```python
from build123d import *

# Parameters (mm, degrees)
BOSS_EXTRUDE1_DEPTH                                 = 8
CBORE_FOR_M3_HEX_SOCKET_HEAD_CAP_SCREW1_D           = 3.4
CBORE_FOR_M3_HEX_SOCKET_HEAD_CAP_SCREW1_CBORE_D     = 6.5
CBORE_FOR_M3_HEX_SOCKET_HEAD_CAP_SCREW1_CBORE_DEPTH = 3.4


with BuildPart() as part:
    # Sketch1 → Boss-Extrude1 (new body)
    with BuildSketch(Plane.XY):
        with BuildLine():
            Line((-27.5, 4), (27.5, 4))
            ThreePointArc((27.5, 4), (31.5, 0), (27.5, -4))
            Line((27.5, -4), (-27.5, -4))
            ThreePointArc((-27.5, -4), (-31.5, 0), (-27.5, 4))
        make_face()
    extrude(amount=BOSS_EXTRUDE1_DEPTH)

    # CBORE for M3 Hex Socket Head Cap Screw1 (through all)
    with Locations(Plane.XY.offset(8)):
        with Locations((-20, 0), (20, 0)):
            CounterBoreHole(CBORE_FOR_M3_HEX_SOCKET_HEAD_CAP_SCREW1_D / 2, CBORE_FOR_M3_HEX_SOCKET_HEAD_CAP_SCREW1_CBORE_D / 2, CBORE_FOR_M3_HEX_SOCKET_HEAD_CAP_SCREW1_CBORE_DEPTH)


solid = part.part
```
Design review of the part built by this model. Coordinates are the model's own, in mm. A direction names the side the tool comes from. Coordinates: 2 decimals unless noted, no trailing zeros. Order: outer loops, then holes, each group sorted by start corner. A loop starts at its lowest first (then second) coordinate and runs counter-clockwise, first axis right, second up. Notation, with made-up numbers: M 31.25,54 L 87.25,54 A19 cw 87.25,59 Z; hole C 33.5,70.5 d5. An arc over 180 degrees is marked long. Answer as a JSON object with one key per item and string values. Group by question number.
1) Add section B-B, the plane y = 0. Write out the cut boundary in (x, z).
2) Wall thickness on L1, parallel to Y at x = -20, z = 6.1; L2, parallel to X at y = 2.5, z = 6.25; L3, parallel to Y at x = 20, z = 2.05: over which ranges is each line inside the solid? List them lowest first.
3) Tool access review of faces 4 (the cylindrical face through (16.753, 0.143, 6.324)), 5 (the cylindrical face through (18.43, -0.65, 2.27)): name each direction out of +Z, -Z, +X, -X, +Y, -Y from which nothing blocks a thin tool from reaching the whole face with its end or side.
4) Add section A-A, the plane x = 20. Write out the cut boundary in (y, z).
5) For pin 1 (4 mm diameter, centred on x = -20, y = 0, fed in from +Z), flat-tipped, find the tip position at first contact; note if it passes through.
6) Add section C-C, the plane z = 3.5. Write out the cut boundary in (x, y), then the cut area to 3 significant figures.
7) Mouldability with a two-part tool opening along X and no side actions: class faces 1 (the cylindrical face through (31.5, 0.1, 3.9)), 2 (the flat face through (21.4, -1.4, 4.6)), 3 (the flat face through (0, 0, 8)) as pulls with the +X half, pulls with the -X half, needs draft (parallel to the pull), parting line crosses it, or undercut.
Computed values:
{
 "1": {"outline": "M -31.5,0 L -21.7,0 L -21.7,4.6 L -23.25,4.6 L -23.25,8 L -31.5,8 Z; M -18.3,0 L 18.3,0 L 18.3,4.6 L 16.75,4.6 L 16.75,8 L -16.75,8 L -16.75,4.6 L -18.3,4.6 Z; M 21.7,0 L 31.5,0 L 31.5,8 L 23.25,8 L 23.25,4.6 L 21.7,4.6 Z"},
 "2": {"L1": "y = -4 to -3.25, 3.25 to 4", "L2": "x = -30.62 to -22.08, -17.92 to 17.92, 22.08 to 30.62", "L3": "y = -4 to -1.7, 1.7 to 4"},
 "3": {"face 4": "+Z", "face 5": "+Z, -Z"},
 "4": {"outline": "M -4,0 L -1.7,0 L -1.7,4.6 L -3.25,4.6 L -3.25,8 L -4,8 Z; M 1.7,0 L 4,0 L 4,8 L 3.25,8 L 3.25,4.6 L 1.7,4.6 Z"},
 "5": {"pin 1": "stops at z = 4.6"},
 "6": {"outline": "M -27.5,-4 L 27.5,-4 A4 ccw 27.5,4 L -27.5,4 A4 ccw Z; hole C -20,0 d3.4; hole C 20,0 d3.4", "area": "472 mm^2"},
 "7": {"face 1": "pulls with the +X half", "face 2": "undercut", "face 3": "needs draft"}
}
